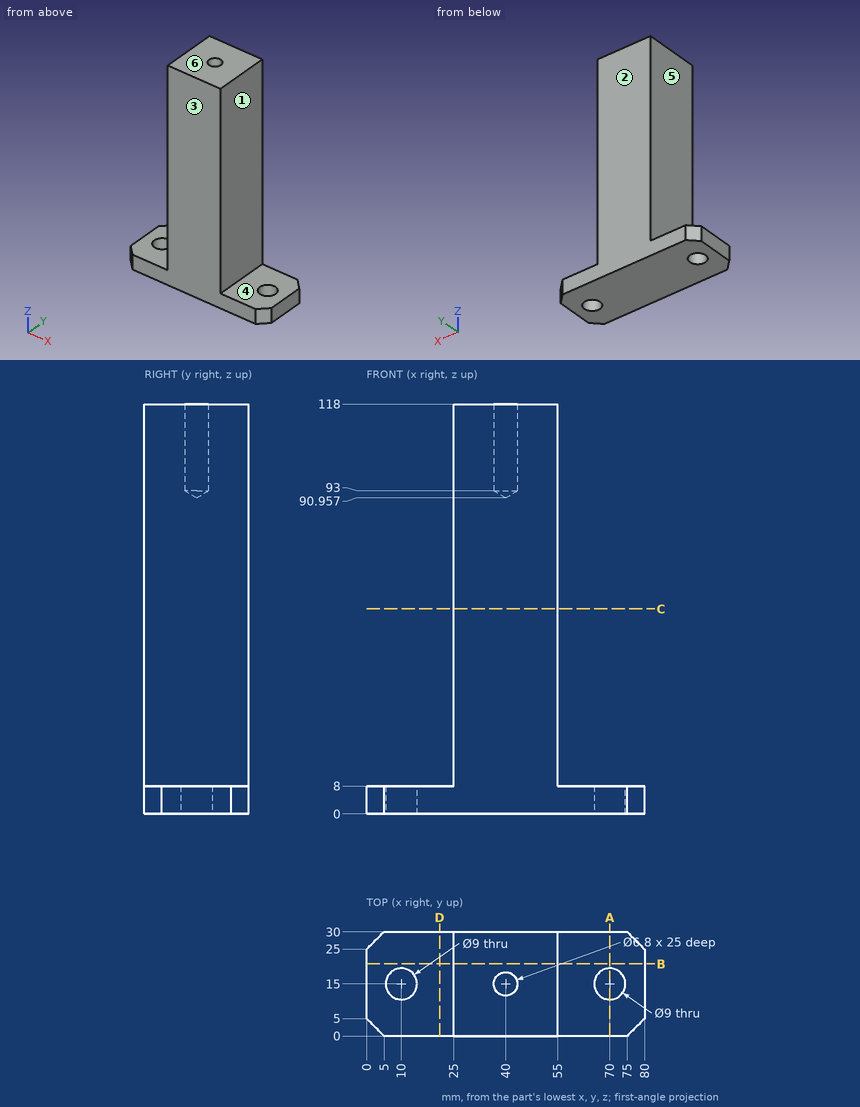
Input: dimensioned drawing with shaded views. Units: mm. Origin: part minimum x, y, z. A direction names the side the tool comes from. Coordinates: 2 decimals unless noted, no trailing zeros. Order: outer loops, then holes, each group sorted by start corner. A loop starts at its lowest first (then second) coordinate and runs counter-clockwise, first axis right, second up.
(1) Access query for the marked faces 4, 5 and 6. Directions: +Z, -Z, +X, -X, +Y, -Y. A direction counts if a zero-diameter tool reaches every point of the face in a straight line with its end or side. Return the directions, or none.
(2) Section query D-D (x = 21). Return the cut outline in (y, z), plus the area to 3 significant figures.
(3) Material intervals for probe 1 along Y at (x, z) = (10, 4); probe 2 along X at (y, z) = (15, 99); probe 3 along X at (y, z) = (24.25, 71), sorted ascending.
(4) Section query B-B (y = 20.75). Return the cut outline in (x, z), plus the area to 3 significant figures.
(5) Draft query along Y for the marked faces 1, 2 and 3. Return one class per face: pulls with the +Y half, pulls with the -Y half, needs draft (parallel to the pull), parting line crosses it, or undercut.
(6) Section query C-C (z = 59). Return the cut outline in (x, y).
(7) First-contact query: pin 1 (5 mm diameter, centred on y = 5, z = 62.5, fed in from -X); pin 2 (5.5 mm diameter, centred on x = 40, y = 15, fed in from +Z); pin 3 (1 mm diameter, centred on y = 9, z = 98.5, fed in from +X). Flat tips, straight axial feed; report the tip coordinate or a pass-through.
(8) Section query A-A (x = 70). Return the cut outline in (y, z).
Solution:
1. face 4: +Z, +X, +Y, -Y
1. face 5: +Z, -X, +Y, -Y
1. face 6: +Z, +X, -X, +Y, -Y
2. outline: (0, 0) - (30, 0) - (30, 8) - (0, 8) - close
2. area: 240 mm2
3. probe 1: y = 0 to 10.5, 19.5 to 30
3. probe 2: x = 25 to 36.6, 43.4 to 55
3. probe 3: x = 25 to 55
4. outline: (0, 0) - (80, 0) - (80, 8) - (55, 8) - (55, 118) - (25, 118) - (25, 8) - (0, 8) - close
4. area: 3,940 mm2
5. face 1: needs draft
5. face 2: pulls with the +Y half
5. face 3: pulls with the -Y half
6. outline: (25, 0) - (55, 0) - (55, 30) - (25, 30) - close
7. pin 1: stops at x = 25
7. pin 2: stops at z = 92.61
7. pin 3: stops at x = 55
8. outline: (0, 0) - (10.5, 0) - (10.5, 8) - (0, 8) - close; (19.5, 0) - (30, 0) - (30, 8) - (19.5, 8) - close
